Design review of the part shown in the three views and the two pictorial views. Dimensions are in mm from the part's minimum x, y and z. A direction names the side the tool comes from. Give positions to 0.01 mm unless a question says otherwise; leave off trailing zeros. Loops run counter-clockwise (first coordinate to the right, second up) from the corner with the lowest first, then second, coordinate; pieces in that order, holes last.
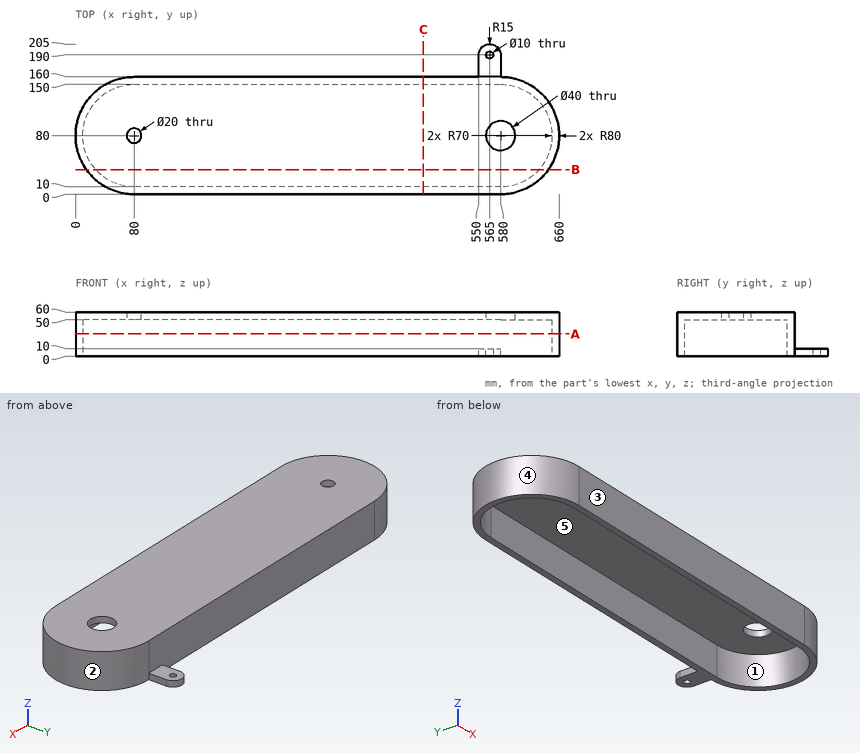
Q1. Draft analysis for pull direction Y (two halves, no side actions). For the marked faces 1, 2 and 3, state which applies: pulls with the +Y half, pulls with the -Y half, needs draft (parallel to the pull), parting line crosses it, or undercut.
Results:
face 1: undercut
face 2: parting line crosses it
face 3: pulls with the -Y half
Q2. Take a section at B-B (y = 33.5). Give the boundary of the cut face in (x, z), plus the area to 3 significant figures.
Results:
outline: (14.9, 0) - (27.68, 0) - (27.68, 50) - (632.32, 50) - (632.32, 0) - (645.1, 0) - (645.1, 60) - (14.9, 60) - close
area: 7,580 mm2
Q3. Take a section at C-C (x = 474.5). Give the boundary of the cut face in (y, z), plus the area to 3 significant figures.
Results:
outline: (0, 0) - (10, 0) - (10, 50) - (150, 50) - (150, 0) - (160, 0) - (160, 60) - (0, 60) - close
area: 2,600 mm2
Q4. Tool access review of the marked faces 4 and 5: name each direction out of +Z, -Z, +X, -X, +Y, -Y from which nothing blocks a thin tool from reaching the whole face with its end or side.
Results:
face 4: +Z, -Z, -X
face 5: -Z
Q5. Wall thickness on line 1 (Y direction, x = 565, z = 3); line 2 (Y direction, x = 479, z = 4); line 3 (X direction, y = 77.5, z = 3.5): over which ranges is each line inside the solid? List them lowest first.
Results:
line 1: y = 0 to 10, 150 to 185, 195 to 205
line 2: y = 0 to 10, 150 to 160
line 3: x = 0.04 to 10.04, 649.96 to 659.96
Q6. Insertion check: pin 1 (13 mm diameter, centred on x = 565, y = 190, fed in from +Z); pin 2 (10 mm diameter, centred on x = 387, z = 13, fed in from +Y); pin 3 (8 mm diameter, centred on y = 168, z = 3.5, fed in from -X). Each pin has a flat end and moves straight along its axis. Give the tip position at first contact, or say it passes through.
Results:
pin 1: stops at z = 10
pin 2: stops at y = 160
pin 3: stops at x = 550
Q7. Take a section at A-A (z = 30.5). Give the boundary of the cut face in (x, y), plus the area to 3 significant figures.
Results:
outline: (80, 0) - (580, 0) arc R80 ccw to (580, 160) - (80, 160) arc R80 ccw to start; hole (80, 10) - (580, 10) arc R70 ccw to (580, 150) - (80, 150) arc R70 ccw to start
area: 14,700 mm2
